Verification items for this drawing (mm, ordinates from the low corner). A direction names the side the tool comes from. Round coordinates to 2 decimals unless told otherwise and drop trailing zeros. Write each loop counter-clockwise with the first axis right and the second up, starting at its lowest first coordinate (ties: lowest second). Pieces come first, ordered by that corner, then holes. Notation, with made-up numbers: (61.5, -4) -> (92.5, -4) arc R15 cw to (92.5, 7) -> close; hole circle Ø4 at (-33, -23.5). An arc over 180 degrees is marked (long way). One line per question, with ' | ' between items.
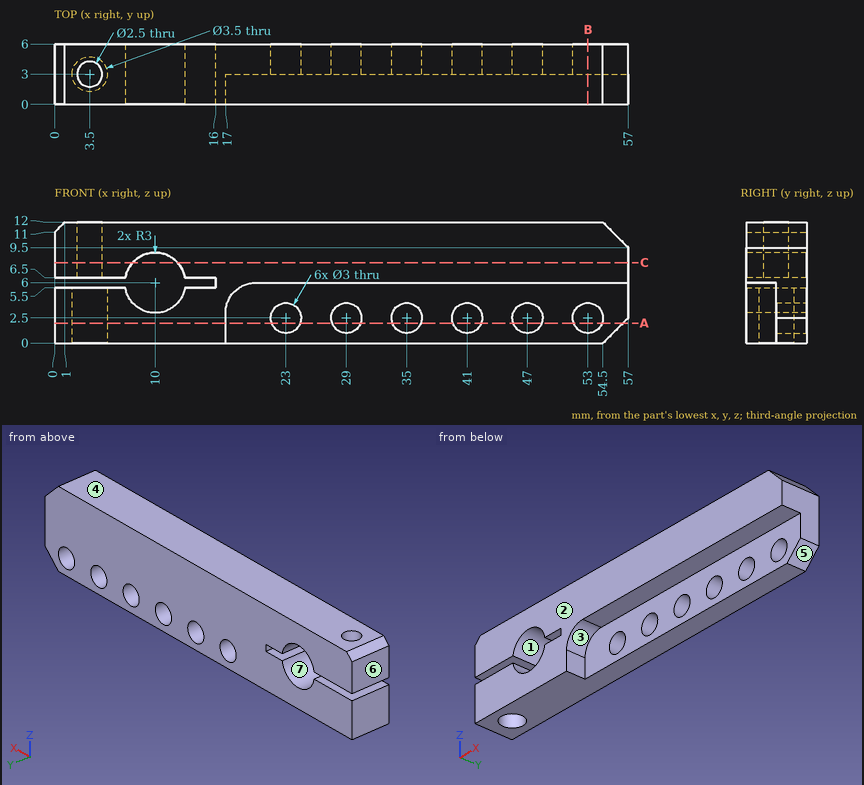
(1) Access from +Z, -Z, +X, -X, +Y, -Y to the whole of each face (thin tool, end or side, straight path). Record for the marked faces 1, 2 and 3.
Resolved:
face 1: +Y, -Y | face 2: +Z, -Z, +X, -X, -Y | face 3: -Z, +X, -Y
(2) Sectioned sample at A-A on z = 2. Count the separate pieces of the cut face and the enclosed holes in it, then the cut area to 3 significant figures.
Resolved:
separate pieces: 7 | enclosed holes: 1 | area: 160 mm2
(3) Sectioned sample at C-C on z = 8. Record the cut outline in (x, y), then the cut area to 3 significant figures.
Resolved:
outline: (0, 0) -> (7.76, 0) -> (7.76, 6) -> (0, 6) -> close; (12.24, 0) -> (57, 0) -> (57, 6) -> (12.24, 6) -> close; hole circle Ø2.5 at (3.5, 3) | area: 310 mm2
(4) Go/stop test with flat-tipped pins: pin 1 (5 mm diameter, centred on x = 29, z = 2.5, fed in from -Y); pin 2 (2.5 mm diameter, centred on y = 1, z = 1.5, fed in from +X); pin 3 (0.8 mm diameter, centred on y = 3, z = 6, fed in from -X). Record where each tip stops, or that it passes through.
Resolved:
pin 1: stops at y = 3 | pin 2: stops at x = 17 | pin 3: stops at x = 16
(5) Draft check along Z on the marked faces 4, 5, 6 and 7. Enter one of: +Z half, -Z half, draft (parallel to the pull), parting line (faces both ways), or undercut.
Resolved:
face 4: +Z half | face 5: -Z half | face 6: draft | face 7: undercut
(6) Sectioned sample at B-B on x = 53. Record the cut outline in (y, z), then the cut area to 3 significant figures.
Resolved:
outline: (0, 6) -> (3, 6) -> (3, 4) -> (6, 4) -> (6, 12) -> (0, 12) -> close; (3, 0) -> (6, 0) -> (6, 1) -> (3, 1) -> close | area: 45.0 mm2
(7) Material ranges on line 1 (X direction, y = 4.2, z = 5); line 2 (X direction, y = 3.8, z = 7.75); line 3 (Z direction, x = 6.5, y = 1.5), recorded low to high.
Resolved:
line 1: x = 0 to 2.23, 4.77 to 7.17, 12.83 to 57 | line 2: x = 0 to 2.54, 4.46 to 7.56, 12.44 to 57 | line 3: z = 0 to 5.5, 6.5 to 12
